Check sheet for the modelled part. Datum: model origin and axes. Units: mm. A direction names the side the tool comes from. Give positions to 0.01 mm unless a question says otherwise; leave off trailing zeros. Order: outer loops, then holes, each group sorted by start corner. A loop starts at its lowest first (then second) coordinate and runs counter-clockwise, first axis right, second up. Notation, with made-up numbers: (68, 43.5) - (73, 43.5) arc R6 ccw to (73, 52.5) - close; hole circle Ø4 at (75, 66.5). An arc over 180 degrees is marked (long way). Answer in a Markdown table with one row per item.
from build123d import *

# Parameters (mm, degrees)
BLOCK_BODY_DEPTH          = 74
BASE_GROOVE_SKETCH_W      = 44
BASE_GROOVE_SKETCH_H      = 6
BASE_GROOVE_44X6_DEPTH    = 94.187982058
BORE_SKETCH_R             = 19
BORE_38_DEPTH             = 15
WALL_WINDOWS_A_SKETCH_W   = 10
WALL_WINDOWS_A_SKETCH_H   = 8
WALL_WINDOWS_A_10X8_DEPTH = 10
WALL_WINDOWS_B_SKETCH_W   = 10
WALL_WINDOWS_B_SKETCH_H   = 8
WALL_WINDOWS_B_10X8_DEPTH = 10


with BuildPart() as part:
    # Block Profile Sketch → Block Body (new body)
    with BuildSketch(Plane.XY):
        Polygon((-21, 0), (21, 0), (21, 38), (8, 38), (8, 16), (-8, 16), (-8, 38), (-21, 38), align=None)
    extrude(amount=-BLOCK_BODY_DEPTH)

    # Base Groove Sketch → Base Groove 44x6 (cut, through all)
    with BuildSketch(Plane(origin=(21, 0, 0), x_dir=(0, 0, -1), z_dir=(1, 0, 0))):
        with Locations((37, 3)):
            Rectangle(BASE_GROOVE_SKETCH_W, BASE_GROOVE_SKETCH_H)
    extrude(amount=-BASE_GROOVE_44X6_DEPTH, mode=Mode.SUBTRACT)

    # Bore Sketch → Bore Ø38 (cut)
    with BuildSketch(Plane(origin=(0, 38, 0), x_dir=(1, 0, 0), z_dir=(0, 1, 0))):
        with Locations((0, 37)):
            Circle(BORE_SKETCH_R)
    extrude(amount=-BORE_38_DEPTH, mode=Mode.SUBTRACT)

    # Wall Windows A Sketch → Wall Windows A 10x8 (cut)
    with BuildSketch(Plane(origin=(-8, 0, 0), x_dir=(0, 0, -1), z_dir=(1, 0, 0))):
        with Locations((10, 29)):
            Rectangle(WALL_WINDOWS_A_SKETCH_W, WALL_WINDOWS_A_SKETCH_H)
        with Locations((64, 29)):
            Rectangle(WALL_WINDOWS_A_SKETCH_W, WALL_WINDOWS_A_SKETCH_H)
    extrude(amount=-WALL_WINDOWS_A_10X8_DEPTH, mode=Mode.SUBTRACT)

    # Wall Windows B Sketch → Wall Windows B 10x8 (cut)
    with BuildSketch(Plane.ZY.offset(-8)):
        with Locations((-64, 29)):
            Rectangle(WALL_WINDOWS_B_SKETCH_W, WALL_WINDOWS_B_SKETCH_H)
        with Locations((-10, 29)):
            Rectangle(WALL_WINDOWS_B_SKETCH_W, WALL_WINDOWS_B_SKETCH_H)
    extrude(amount=-WALL_WINDOWS_B_10X8_DEPTH, mode=Mode.SUBTRACT)


solid = part.part
(1) Mould release check, pull along Z, two halves, no side actions. Record for faces 1 (the flat face through (13, 29, -15)), 2 (the flat face through (21, 19, -36)): pulls with the +Z half, pulls with the -Z half, needs draft (parallel to the pull), parting line crosses it, or undercut.
Geometry says:
| item | result |
|---|---|
| face 1 | undercut |
| face 2 | needs draft |
(2) Cross-section at B-B, the plane z = -68. Record the cut outline in (x, y), then the cut area to 3 significant figures.
Geometry says:
| item | result |
|---|---|
| outline | (-21, 0) - (21, 0) - (21, 38) - (8, 38) - (8, 33) - (18, 33) - (18, 25) - (8, 25) - (8, 16) - (-8, 16) - (-8, 25) - (-18, 25) - (-18, 33) - (-8, 33) - (-8, 38) - (-21, 38) - close |
| area | 1,080 mm² |
(3) Access from +Z, -Z, +X, -X, +Y, -Y to the whole of each face (thin tool, end or side, straight path). Record for faces 3 (the flat face through (-13, 25, -10)), 4 (the flat face through (0, 0, -7)), 5 (the cylindrical face through (-19, 31, -37)), 6 (the flat face through (-21, 19, -36)), 7 (the flat face through (0, 16, -36)).
Geometry says:
| item | result |
|---|---|
| face 3 | none |
| face 4 | +Z, -Z, +X, -X, -Y |
| face 5 | +Y |
| face 6 | +Z, -Z, -X, +Y, -Y |
| face 7 | +Z, -Z, +Y |
(4) Thickness scan on L1, parallel to Y at x = 10, z = -6.5; L2, parallel to Z at x = -14, y = 32; L3, parallel to Z at x = 11, y = 30. Record the ranges inside material, lowest first.
Geometry says:
| item | result |
|---|---|
| L1 | 0 to 25, 33 to 38 |
| L2 | -74 to -69, -59 to -49.85, -24.15 to -15, -5 to 0 |
| L3 | -74 to -69, -59 to -52.49, -21.51 to -15, -5 to 0 |
(5) Cross-section at A-A, the plane y = 31.5. Record the cut outline in (x, z).
Geometry says:
| item | result |
|---|---|
| outline | (-21, -74) - (-8, -74) - (-8, -69) - (-18, -69) - (-18, -59) - (-8, -59) - (-8, -54.23) arc R19 cw to (-8, -19.77) - (-8, -15) - (-18, -15) - (-18, -5) - (-8, -5) - (-8, 0) - (-21, 0) - close; (8, -74) - (21, -74) - (21, 0) - (8, 0) - (8, -5) - (18, -5) - (18, -15) - (8, -15) - (8, -19.77) arc R19 cw to (8, -54.23) - (8, -59) - (18, -59) - (18, -69) - (8, -69) - close |
(6) Cross-section at D-D, the plane y = 19. Record the cut outline in (x, z), then the cut area to 3 significant figures.
Geometry says:
| item | result |
|---|---|
| outline | (-21, -74) - (-8, -74) - (-8, 0) - (-21, 0) - close; (8, -74) - (21, -74) - (21, 0) - (8, 0) - close |
| area | 1,920 mm² |
(7) Gauge pin test, flat ends, axial feed: P1, Ø3.5, axis at x = 15, z = -45, coming from the +Y side; P2, Ø2, axis at x = -16, y = 32.5, coming from the +Z side; P3, Ø1.5, axis at x = -4.5, z = -27.5, coming from the +Y side. Record the tip position at first contact, or that the pin passes through.
Geometry says:
| item | result |
|---|---|
| P1 | y = 23 |
| P2 | z = 0 |
| P3 | y = 16 |
(8) Cross-section at C-C, the plane x = 3. Record the cut outline in (y, z).
Geometry says:
| item | result |
|---|---|
| outline | (0, -74) - (16, -74) - (16, 0) - (0, 0) - (0, -15) - (6, -15) - (6, -59) - (0, -59) - close |
